Print and shaded views of the part. All mm, measured from the part's lowest x, y and z. A direction names the side the tool comes from. Give positions to 0.01 mm unless a question says otherwise; leave off trailing zeros. Write each loop counter-clockwise with the first axis right and the second up, starting at its lowest first coordinate (ties: lowest second). Pieces come first, ordered by that corner, then holes.
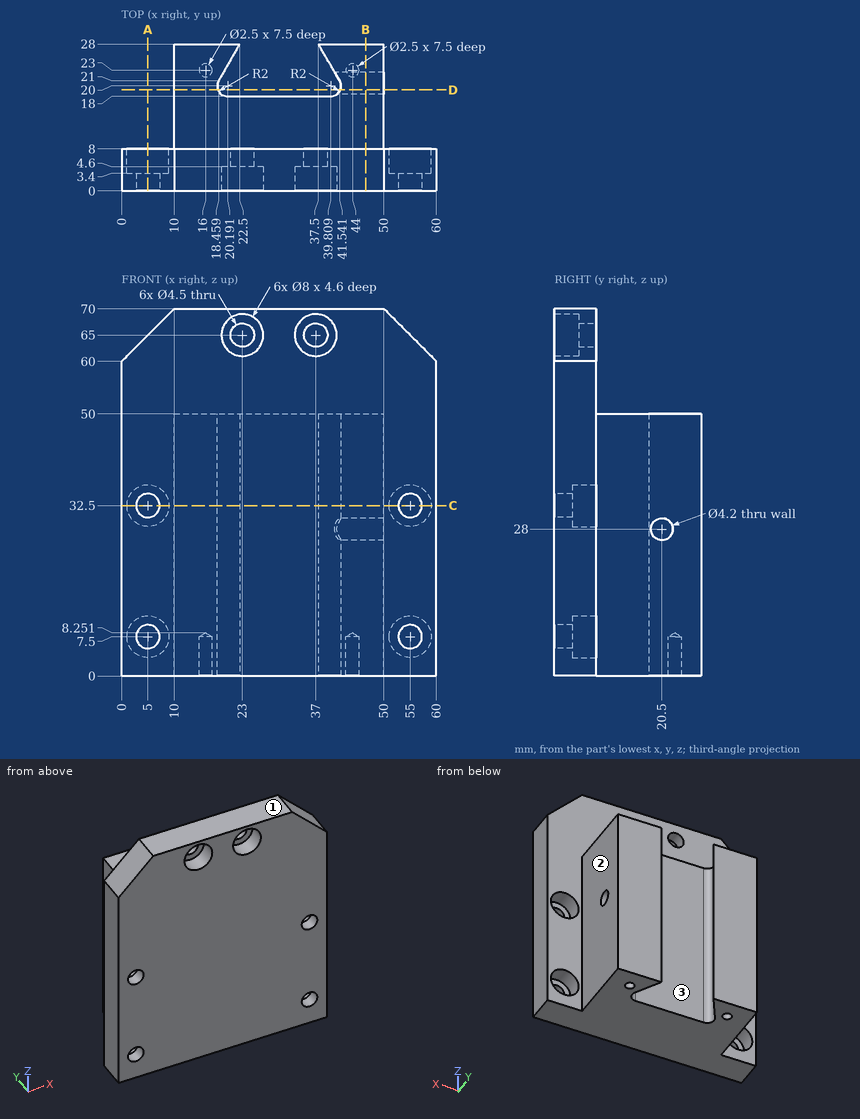
1. 3-axis set-ups, long thin cutter, end or side, ignore diameter. For the marked faces 1, 2 and 3: which of +Z, -Z, +X, -X, +Y, -Y reach the whole face in a straight line?
2. Saw through at A-A on x = 5. Give the cut face in (y, z), plus the area to 3 significant figures.
3. Drop flat-ended pins along their axis: pin 1 (2.5 mm diameter, centred on x = 6, z = 34.5, fed in from +Y); pin 2 (5 mm diameter, centred on x = 5, z = 32.5, fed in from -Y); pin 3 (1 mm diameter, centred on y = 9, z = 12, fed in from +X); pin 4 (3 mm diameter, centred on y = 23, z = 33.5, fed in from -X). Give the stop position or say it passes through.
4. Drill centre lines: line 1 along X through (y, z) = (20, 5); line 2 along Z through (x, y) = (55.5, 5); line 3 along Z through (x, y) = (54.5, 5.25). Where is each one in solid material? Low to high.
5. Saw through at B-B on x = 46.5. Give the cut face in (y, z).
6. Saw through at C-C on z = 32.5. Count the separate pieces of the cut face and the enclosed holes in it.
7. Saw through at D-D on y = 19.25. Give the cut face in (x, z).
Outcome:
1. face 1: +Z, +X, -X, +Y, -Y
1. face 2: +Z, -Z, +X, +Y
1. face 3: +Z, -Z
2. outline: (0, 0) - (8, 0) - (8, 3.5) - (3.4, 3.5) - (3.4, 5.25) - (0, 5.25) - close; (0, 9.75) - (3.4, 9.75) - (3.4, 11.5) - (8, 11.5) - (8, 28.5) - (3.4, 28.5) - (3.4, 30.25) - (0, 30.25) - close; (0, 34.75) - (3.4, 34.75) - (3.4, 36.5) - (8, 36.5) - (8, 65) - (0, 65) - close
2. area: 416 mm2
3. pin 1: stops at y = 3.4
3. pin 2: stops at y = 0
3. pin 3: stops at x = 50
3. pin 4: stops at x = 10
4. line 1: x = 10 to 18.19, 41.81 to 50
4. line 2: z = 0 to 3.53, 11.47 to 28.53, 36.47 to 64.5
4. line 3: z = 0 to 3.53, 11.47 to 28.53, 36.47 to 65.5
5. outline: (0, 0) - (28, 0) - (28, 50) - (8, 50) - (8, 70) - (0, 70) - close; hole circle Ø4.2 at (20.5, 28)
6. separate pieces: 3
6. enclosed holes: 0
7. outline: (10, 0) - (18.34, 0) - (18.34, 50) - (10, 50) - close; (41.66, 0) - (50, 0) - (50, 26.31) - (41.66, 26.31) - close; (41.66, 29.69) - (50, 29.69) - (50, 50) - (41.66, 50) - close
